Design review of the part built by this model. Coordinates are the model's own, in mm. A direction names the side the tool comes from. Coordinates: 2 decimals unless noted, no trailing zeros. Write each loop counter-clockwise with the first axis right and the second up, starting at its lowest first coordinate (ties: lowest second). Pieces come first, ordered by that corner, then holes. Notation, with made-up numbers: M 47.25,47 L 91.25,47 A19 ccw 91.25,67 Z; hole C 57,4 d10. An arc over 180 degrees is marked long. Return JSON: item names as keys, results as strings. Group by question number.
```python
from build123d import *

# Parameters (mm, degrees)
SKETCH_1_W                     = 62
SKETCH_1_H                     = 62
EXTRUDE_1_DEPTH                = 6
SKETCH_2_R                     = 16
CUT_EXTRUDE_1_DEPTH            = 46.453272709
HOLE_WIZARD_M5_1_D             = 4.2
SKETCH_11_R                    = 25
CUT_EXTRUDE_2_DEPTH            = 7
HOLE_WIZARD_M5_1_2_D           = 5.5
HOLE_WIZARD_M5_1_2_CBORE_D     = 10.1
HOLE_WIZARD_M5_1_2_CBORE_DEPTH = 5.4
CHAMFER_1_SIZE                 = 2
SKETCH_13_R                    = 19.2
SKETCH_13_R_2                  = 16.8
CUT_EXTRUDE_3_DEPTH            = 1.5


with BuildPart() as part:
    # 草图1 → 凸台-拉伸1 (new, symmetric)
    with BuildSketch(Plane.XY):
        Rectangle(SKETCH_1_W, SKETCH_1_H)
    extrude(amount=EXTRUDE_1_DEPTH, both=True)

    # 草图2 → 切除-拉伸1 (cut, through all)
    with BuildSketch(Plane.XY.offset(6)):
        Circle(SKETCH_2_R)
    extrude(amount=-CUT_EXTRUDE_1_DEPTH, mode=Mode.SUBTRACT)

    # Hole Wizard M5 _1 (through all)
    with Locations(Plane(origin=(0, 0, -6), x_dir=(1, 0, 0), z_dir=(0, 0, -1))):
        with Locations((-24.748737342, -24.748737342), (24.748737342, -24.748737342), (-24.748737342, 24.748737342), (24.748737342, 24.748737342)):
            Hole(HOLE_WIZARD_M5_1_D / 2)

    # 草图11 → 切除-拉伸2 (cut)
    with BuildSketch(Plane(origin=(0, 0, -6), x_dir=(-1, 0, 0), z_dir=(0, 0, -1))):
        Circle(SKETCH_11_R)
    extrude(amount=-CUT_EXTRUDE_2_DEPTH, mode=Mode.SUBTRACT)

    # Hole Wizard M5 _1 2 (through all)
    with Locations(Plane(origin=(0, 0, -6), x_dir=(-1, 0, 0), z_dir=(0, 0, -1))):
        with Locations((-25, 16.5), (25, 16.5), (25, -16.5), (-25, -16.5)):
            CounterBoreHole(HOLE_WIZARD_M5_1_2_D / 2, HOLE_WIZARD_M5_1_2_CBORE_D / 2, HOLE_WIZARD_M5_1_2_CBORE_DEPTH)

    # 倒角1
    chamfer_1_edges = [part.edges().sort_by_distance(p)[0] for p in [
        (31, -31, 0),
        (-31, -31, 0),
        (-31, 31, 0),
        (31, 31, 0),
    ]]
    chamfer(chamfer_1_edges, length=CHAMFER_1_SIZE)

    # 草图13 → 切除-拉伸3 (cut)
    with BuildSketch(Plane(origin=(0, 0, 1), x_dir=(-1, 0, 0), z_dir=(0, 0, -1))):
        Circle(SKETCH_13_R)
        Circle(SKETCH_13_R_2, mode=Mode.SUBTRACT)
    extrude(amount=-CUT_EXTRUDE_3_DEPTH, mode=Mode.SUBTRACT)


solid = part.part
```
Item 1: For line 1 (Y direction, x = 25, z = 2.75); line 2 (Y direction, x = 0, z = 2.05); line 3 (Z direction, x = 19, y = -2.5), list the stretches that pass through material, from the lowest coordinate up.
Item 2: For pin 1 (7 mm diameter, centred on x = 25, y = 16.5, fed in from -Z); pin 2 (19 mm diameter, centred on x = -8.5, y = 9.5, fed in from -Z); pin 3 (1 mm diameter, centred on x = -4.5, y = 14.5, fed in from +Z), all flat-tipped, find the tip position at first contact; note any pin that passes through.
Item 3: Add section C-C (z = -3.5). Write out the cut boundary in (x, y).
Item 4: Machinability: for faces 1 (the flat face through (0, -31, 0)), 2 (the flat face through (-15, -6, 1)), which of the approach directions +Z, -Z, +X, -X, +Y, -Y give a long, thin tool a straight path to every point of the face, cutting with its end or side? Answer none if there is none.
Item 5: Add section D-D (x = 24). Count the separate pieces of the cut face and the enclosed holes in it, plus the area to 3 significant figures.
Item 6: The part is to be moulded in two halves that separate along Y. For faces 3 (the cylindrical face through (29.33, -19.1, -3.34)), 4 (the flat face through (-31, 0, 0)), 5 (the flat face through (30, 30, 0)), say which applies: pulls with the +Y half, pulls with the -Y half, needs draft (parallel to the pull), parting line crosses it, or undercut.
Item 7: Add section A-A (y = 0). Write out the cut boundary in (x, z).
Geometry check:
{
 "1": {"line 1": "-31 to -26.83, -22.66 to -19.25, -13.75 to 13.75, 19.25 to 22.66, 26.83 to 31", "line 2": "-31 to -19.2, -16.8 to -16, 16 to 16.8, 19.2 to 31", "line 3": "2.5 to 6"},
 "2": {"pin 1": "z = -0.6", "pin 2": "z = 1", "pin 3": "through"},
 "3": {"outline": "M -31,-29 L -29,-31 L 29,-31 L 31,-29 L 31,29 L 29,31 L -29,31 L -31,29 Z; hole C -24.75,-24.75 d4.2; hole C -24.75,24.75 d4.2; hole M -21.34,-13.02 A5.05 ccw long -20.36,-14.51 A25 ccw 20.36,-14.51 A5.05 ccw long 21.34,-13.02 A25 ccw 21.34,13.02 A5.05 ccw long 20.36,14.51 A25 ccw -20.36,14.51 A5.05 ccw long -21.34,13.02 A25 ccw Z; hole C 24.75,-24.75 d4.2; hole C 24.75,24.75 d4.2"},
 "4": {"face 1": "+Z, -Z, +X, -X, -Y", "face 2": "-Z"},
 "5": {"separate pieces": "5", "enclosed holes": "0", "area": "377 mm^2"},
 "6": {"face 3": "undercut", "face 4": "needs draft", "face 5": "pulls with the +Y half"},
 "7": {"outline": "M -31,-6 L -25,-6 L -25,1 L -19.2,1 L -19.2,2.5 L -16.8,2.5 L -16.8,1 L -16,1 L -16,6 L -31,6 Z; M 16,1 L 16.8,1 L 16.8,2.5 L 19.2,2.5 L 19.2,1 L 25,1 L 25,-6 L 31,-6 L 31,6 L 16,6 Z"}
}
